Design review of the part built by this model. Coordinates are the model's own, in mm. Face numbers are marked on the shaded views. Give positions to 0.01 mm unless a question says otherwise; leave off trailing zeros. Write each loop counter-clockwise with the first axis right and the second up, starting at its lowest first coordinate (ties: lowest second). Pieces come first, ordered by that corner, then holes. Notation, with made-up numbers: M 82.5,11.25 L 113.5,11.25 A26 ccw 113.5,35.25 Z; hole C 51.25,15.25 d9. An arc over 180 degrees is marked long. Answer in a Markdown table with one row per item.
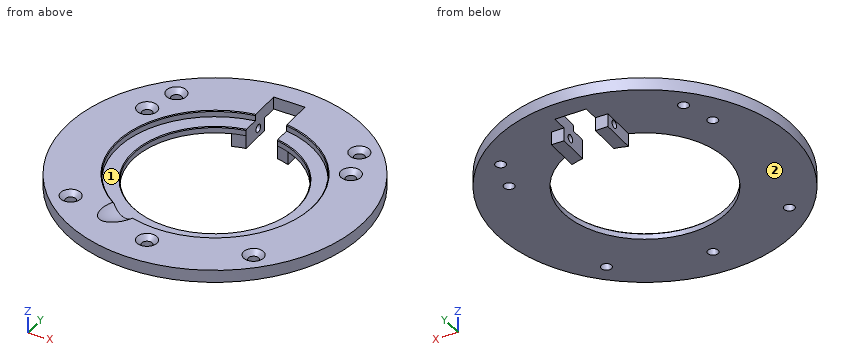
```python
from build123d import *

# Parameters (mm, degrees)
SKETCH_1_R               = 95
SKETCH_1_R_2             = 52.5
EXTRUDE_1_DEPTH          = 8
SKETCH_3_R               = 62.5
CUT_EXTRUDE_1_DEPTH      = 4
PATTERN_CIRCULAR_1_COUNT = 3
PATTERN_CIRCULAR_2_COUNT = 4
SKETCH_7_W               = 20
SKETCH_7_H               = 39
CUT_EXTRUDE_2_DEPTH      = 10
EXTRUDE_START            = 8.5
EXTRUDE_2_DEPTH          = 8.5
SKETCH_9_R               = 2.5
CUT_EXTRUDE_3_DEPTH      = 148.87241122
CHAMFER_1_SIZE           = 0.5


with BuildPart() as part:
    # 草图1 → 凸台-拉伸1 (new body)
    with BuildSketch(Plane.XY):
        Circle(SKETCH_1_R)
        Circle(SKETCH_1_R_2, mode=Mode.SUBTRACT)
    extrude(amount=EXTRUDE_1_DEPTH)

    # 草图3 → 切除-拉伸1 (cut)
    with BuildSketch(Plane.XY.offset(8)):
        Circle(SKETCH_3_R)
    extrude(amount=-CUT_EXTRUDE_1_DEPTH, mode=Mode.SUBTRACT)

    # 草图5 → 打孔尺寸(%根据)内六角花形半沉头螺钉的类型1 (revolve, cut)
    with BuildSketch(Plane(origin=(0, -75, 8), x_dir=(0, -1, 0), z_dir=(1, 0, 0))):
        Polygon((0, 0), (0, 26.482840043), (3.3, 24.5), (3.3, 3.1), (6.4, 0), align=None)
    hole_wizard_1 = revolve(axis=Axis((0, -75, 14.35), (0, 0, -1)), mode=Mode.SUBTRACT)

    # 草图6 → 打孔尺寸(%根据)内六角花形半沉头螺钉的类型2 (revolve, cut)
    with BuildSketch(Plane(origin=(-58.336309448, -58.336309448, 8), x_dir=(0, -1, 0), z_dir=(1, 0, 0))):
        Polygon((0, 0), (0, 26.482840043), (3.3, 24.5), (3.3, 3.1), (6.4, 0), align=None)
    hole_wizard_2 = revolve(axis=Axis((-58.336309448, -58.336309448, 14.35), (0, 0, -1)), mode=Mode.SUBTRACT)

    # 阵列(圆周)1: 打孔尺寸(%根据)内六角花形半沉头螺钉的类型1 ×3 about axis
    pattern_circular_1_axis = Axis((0, 0, 0), (0, 0, 1))
    for i in range(1, PATTERN_CIRCULAR_1_COUNT):
        add(hole_wizard_1.rotate(pattern_circular_1_axis, i * 360 / PATTERN_CIRCULAR_1_COUNT), mode=Mode.SUBTRACT)

    # 阵列(圆周)2: 打孔尺寸(%根据)内六角花形半沉头螺钉的类型2 ×4 about axis
    pattern_circular_2_axis = Axis((0, 0, 0), (0, 0, 1))
    for i in range(1, PATTERN_CIRCULAR_2_COUNT):
        add(hole_wizard_2.rotate(pattern_circular_2_axis, i * 360 / PATTERN_CIRCULAR_2_COUNT), mode=Mode.SUBTRACT)

    # 草图7 → 切除-拉伸2 (cut)
    with BuildSketch(Plane.XY.offset(8)):
        with Locations((0, 62.5)):
            Rectangle(SKETCH_7_W, SKETCH_7_H)
    extrude(amount=-CUT_EXTRUDE_2_DEPTH, mode=Mode.SUBTRACT)

    # 草图8 → 凸台-拉伸2 (add)
    with BuildSketch(Plane(origin=(0, 0, 0), x_dir=(-1, 0, 0), z_dir=(0, 0, -1)).offset(EXTRUDE_START)):
        with BuildLine():
            Line((10, 72), (18, 72))
            Line((18, 72), (18, 49.317846668))
            ThreePointArc((18, 49.317846668), (14.04397312, 50.586725719), (10, 51.53882032))
            Line((10, 51.53882032), (10, 72))
        make_face()
        with BuildLine():
            Line((-10, 72), (-18, 72))
            Line((-18, 72), (-18, 49.317846668))
            ThreePointArc((-18, 49.317846668), (-14.04397312, 50.586725719), (-10, 51.53882032))
            Line((-10, 51.53882032), (-10, 72))
        make_face()
    extrude(amount=-EXTRUDE_2_DEPTH)

    # 草图9 → 切除-拉伸3 (cut, through all)
    with BuildSketch(Plane(origin=(18, 0, 0), x_dir=(0, 0, -1), z_dir=(1, 0, 0))):
        with Locations(Location((3, 65, 0), (0, 0, 90))):
            Circle(SKETCH_9_R)
    extrude(amount=-CUT_EXTRUDE_3_DEPTH, mode=Mode.SUBTRACT)

    # 倒角1
    chamfer_1_edges = [part.edges().sort_by_distance(p)[0] for p in [
        (0, -52.5, 4),
        (0, -62.5, 8),
    ]]
    chamfer(chamfer_1_edges, length=CHAMFER_1_SIZE)

    # 草图12 → 切除-旋转1 (revolve, cut)
    with BuildSketch(Plane(origin=(0, 0, 0), x_dir=(0, 0, -1), z_dir=(-0.9063077870366526, 0.42261826174069383, 0))):
        with BuildLine():
            Line((-17.5, 88), (-17.5, 38))
            ThreePointArc((-17.5, 38), (-4.054529719, 63), (-17.5, 88))
        make_face()
    revolve(axis=Axis((-37.190407033, -79.755085259, 17.5), (0.4226182617406939, 0.9063077870366525, 0)), mode=Mode.SUBTRACT)


solid = part.part
```
1) The part is to be moulded in two halves that separate along Y. For the marked faces 1 and 2, say which applies: released by +Y, released by -Y, zero draft, split by the parting line, or undercut.
Geometry says:
| item | result |
|---|---|
| face 1 | undercut |
| face 2 | zero draft |
2) Insertion check: P1, Ø8, axis at y = 60, z = -1.5, coming from the +X side; P2, Ø2.5, axis at y = 62, z = -5, coming from the +X side; P3, Ø3, axis at y = 65, z = -3, coming from the +X side; P4, Ø8.5, axis at x = 0, y = -75, coming from the +Z side. Each pin has a flat end and moves straight along its axis. Give the tip position at first contact, or say it passes through.
Geometry says:
| item | result |
|---|---|
| P1 | x = 76.53 |
| P2 | x = 18 |
| P3 | through |
| P4 | z = 5.85 |
3) Add section D-D (x = 75). Write out the cut boundary in (y, z), and give its area (3 significant figures).
Geometry says:
| item | result |
|---|---|
| outline | M -58.31,0 L 58.31,0 L 58.31,8 L -58.31,8 Z |
| area | 933 mm^2 |
4) Add section A-A (x = 0). Write out the cut boundary in (y, z).
Geometry says:
| item | result |
|---|---|
| outline | M -95,0 L -78.3,0 L -78.3,4.9 L -81.4,8 L -95,8 Z; M -71.7,0 L -52.5,0 L -52.5,3.5 L -53,4 L -62.5,4 L -62.5,7.5 L -63,8 L -68.6,8 L -71.7,4.9 Z; M 82,0 L 95,0 L 95,8 L 82,8 Z |
5) To check wall thickness, follow probe 1 along Y at (x, z) = (0, 6); probe 2 along Z at (x, y) = (-12.5, 65); probe 3 along Z at (x, y) = (13, 85.5). State the ranges of each line that lie inside material, in increasing order. Write a range as [from, to].
Geometry says:
| item | result |
|---|---|
| probe 1 | [-95, -79.4], [-70.6, -62.5], [82, 95] |
| probe 2 | [-8.5, -5.5], [-0.5, 8] |
| probe 3 | [0, 8] |
6) Add section B-B (z = -3). Write out the cut boundary in (x, y).
Geometry says:
| item | result |
|---|---|
| outline | M -18,49.32 A52.5 cw -10,51.54 L -10,62.5 L -18,62.5 Z; M -18,67.5 L -10,67.5 L -10,72 L -18,72 Z; M 10,51.54 A52.5 cw 18,49.32 L 18,62.5 L 10,62.5 Z; M 10,67.5 L 18,67.5 L 18,72 L 10,72 Z |
7) Add section C-C (y = -75). Write out the cut boundary in (x, z).
Geometry says:
| item | result |
|---|---|
| outline | M -58.31,0 L -3.3,0 L -3.3,4.9 L -6.4,8 L -58.31,8 Z; M 3.3,0 L 58.31,0 L 58.31,8 L 6.4,8 L 3.3,4.9 Z |
